The listing builds one solid part. Answer for the finished solid, in the listing's coordinates (mm). Face numbers are marked on the shaded views. A direction names the side the tool comes from. Give positions to 0.01 mm unless a question says otherwise; leave off trailing zeros. Write each loop counter-clockwise with the first axis right and the second up, starting at its lowest first coordinate (ties: lowest second). Pieces come first, ordered by that corner, then holes. Notation, with made-up numbers: (8, 49.5) - (65, 49.5) arc R25 cw to (65, 73.5) - close; hole circle Ø4 at (71.25, -35.75). An arc over 180 degrees is marked (long way). Return JSON: item names as keys, results as strings.
from build123d import *

# Parameters (mm, degrees)
SKETCH1_R           = 2.25
SKETCH1_R_2         = 3
BOSS_EXTRUDE1_DEPTH = 3
FILLET1_R           = 3
CHAMFER1_SIZE       = 3
CHAMFER2_SIZE       = 1


with BuildPart() as part:
    # Sketch1 → Boss-Extrude1 (new, symmetric)
    with BuildSketch(Plane.XY):
        Polygon((0, 0), (-55, 0), (-55, 8), (-10, 8), (-10, 24), (0, 24), align=None)
        with Locations((-51, 4)):
            Circle(SKETCH1_R, mode=Mode.SUBTRACT)
        with Locations((-34, 4)):
            Circle(SKETCH1_R, mode=Mode.SUBTRACT)
        with Locations((-5, 19)):
            Circle(SKETCH1_R_2, mode=Mode.SUBTRACT)
    extrude(amount=BOSS_EXTRUDE1_DEPTH, both=True)

    # Fillet1
    fillet1_edges = [part.edges().sort_by_distance(p)[0] for p in [
        (-10, 8, 0),
    ]]
    fillet(fillet1_edges, radius=FILLET1_R)

    # Chamfer1
    chamfer1_edges = [part.edges().sort_by_distance(p)[0] for p in [
        (0, 0, 0),
    ]]
    chamfer(chamfer1_edges, length=CHAMFER1_SIZE)

    # Chamfer2
    chamfer2_edges = [part.edges().sort_by_distance(p)[0] for p in [
        (-55, 0, 0),
        (-55, 8, 0),
        (-10, 24, 0),
        (0, 24, 0),
    ]]
    chamfer(chamfer2_edges, length=CHAMFER2_SIZE)


solid = part.part
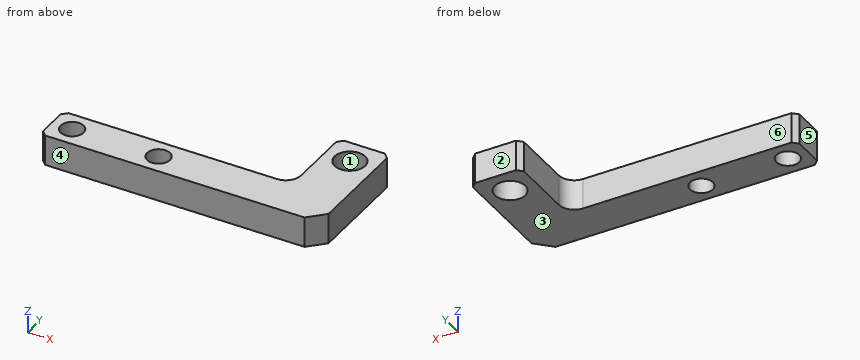
Item 1: Flat-ended cylindrical pins translate along their axes: P1, Ø3, axis at y = 19, z = 0, coming from the -X side; P2, Ø1.5, axis at x = -47.5, z = 0.5, coming from the +Y side. Find the tip coordinate at first contact, or state that the pin passes through.
Answer below:
{"P1": "stops at x = -10", "P2": "stops at y = 8"}
Item 2: A cutting plane is placed at C-C on y = 2.5. Determine the outline of the cut face in (x, z).
Answer below:
{"outline": "(-55, -3) - (-52.68, -3) - (-52.68, 3) - (-55, 3) - close; (-49.32, -3) - (-35.68, -3) - (-35.68, 3) - (-49.32, 3) - close; (-32.32, -3) - (-0.5, -3) - (-0.5, 3) - (-32.32, 3) - close"}
Item 3: Consider L1, parallel to Y at x = -34, z = 0.85; L2, parallel to X at y = 15, z = 0.75; L3, parallel to X at y = 3.5, z = -1.75. Determine where each line is inside the solid, lowest interval first.
Answer below:
{"L1": "y = 0 to 1.75, 6.25 to 8", "L2": "x = -10 to 0", "L3": "x = -55 to -53.19, -48.81 to -36.19, -31.81 to 0"}
Item 4: A cutting plane is placed at A-A on x = -5. Determine the outline of the cut face in (y, z), then the cut area to 3 significant figures.
Answer below:
{"outline": "(0, -3) - (16, -3) - (16, 3) - (0, 3) - close; (22, -3) - (24, -3) - (24, 3) - (22, 3) - close", "area": "108 mm²"}
Item 5: A cutting plane is placed at D-D on y = 21.25. Determine the outline of the cut face in (x, z), then the cut area to 3 significant figures.
Answer below:
{"outline": "(-10, -3) - (-6.98, -3) - (-6.98, 3) - (-10, 3) - close; (-3.02, -3) - (0, -3) - (0, 3) - (-3.02, 3) - close", "area": "36.2 mm²"}
Item 6: A cutting plane is placed at B-B on z = 2. Determine the outline of the cut face in (x, y), then the cut area to 3 significant figures.
Answer below:
{"outline": "(-55, 1) - (-54, 0) - (-3, 0) - (0, 3) - (0, 23) - (-1, 24) - (-9, 24) - (-10, 23) - (-10, 11) arc R3 cw to (-13, 8) - (-54, 8) - (-55, 7) - close; hole circle Ø4.5 at (-51, 4); hole circle Ø4.5 at (-34, 4); hole circle Ø6 at (-5, 19)", "area": "535 mm²"}
Item 7: The mould has two halves that part along Y. Classify the marked faces 1, 2, 3 and 4: +Y half, -Y half, draft (parallel to the pull), parting line (faces both ways), or undercut.
Answer below:
{"face 1": "undercut", "face 2": "+Y half", "face 3": "draft", "face 4": "-Y half"}
Item 8: For the marked faces 5 and 6, determine the directions among +Z, -Z, +X, -X, +Y, -Y from which every point of the face is accessible in a straight line to the end or side of a thin tool.
Answer below:
{"face 5": "+Z, -Z, -X, +Y, -Y", "face 6": "+Z, -Z, -X, +Y"}
